Read the model definition and answer for the solid it produces. Units are mm, in the model's axes. Face numbers are marked on the shaded views. Give positions to 0.01 mm unless a question says otherwise; leave off trailing zeros. Order: outer loops, then holes, each group sorted by start corner. A loop starts at its lowest first (then second) coordinate and runs counter-clockwise, first axis right, second up. Notation, with made-up numbers: (46, -5.5) - (99, -5.5) arc R20 ccw to (99, 3.5) - close; hole circle Ø10 at (53.25, 16.25). An arc over 180 degrees is marked (long way). Answer as CSV lines item,"result". Start each with the question number.
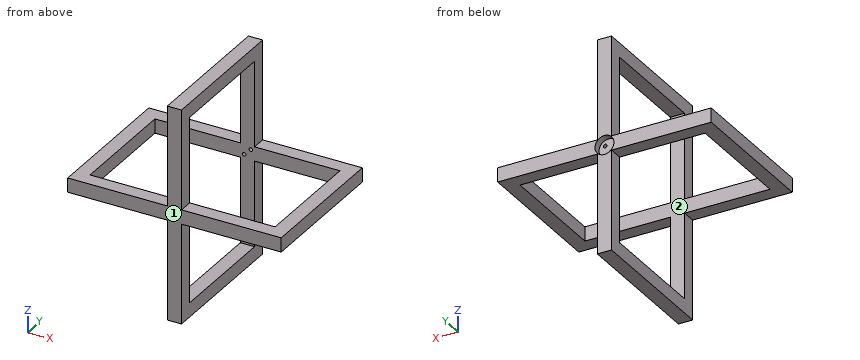
from build123d import *

# Parameters (mm, degrees)
SKETCH1_W                        = 900
SKETCH1_H                        = 600
SKETCH1_W_2                      = 780
SKETCH1_H_2                      = 480
BOSS_EXTRUDE1_DEPTH              = 30
SKETCH2_W                        = 900
SKETCH2_H                        = 600
SKETCH2_W_2                      = 780
SKETCH2_H_2                      = 480
BOSS_EXTRUDE2_DEPTH              = 30
SKETCH3_R                        = 40
CUT_EXTRUDE1_DEPTH               = 30
BLIND_DOWEL_HOLE_0_SIZE_MM_D     = 15
BLIND_DOWEL_HOLE_0_SIZE_MM_DEPTH = 100
BLIND_DOWEL_HOLE_0_SIZE_MM_TIP   = 4.506454643


with BuildPart() as part:
    # Sketch1 → Boss-Extrude1 (new, symmetric)
    with BuildSketch(Plane.XY):
        Rectangle(SKETCH1_W, SKETCH1_H)
        Rectangle(SKETCH1_W_2, SKETCH1_H_2, mode=Mode.SUBTRACT)
    extrude(amount=BOSS_EXTRUDE1_DEPTH, both=True)

    # Sketch2 → Boss-Extrude2 (add, symmetric)
    with BuildSketch(Plane(origin=(0, 0, 0), x_dir=(0, 0, -1), z_dir=(1, 0, 0))):
        Rectangle(SKETCH2_W, SKETCH2_H)
        Rectangle(SKETCH2_W_2, SKETCH2_H_2, mode=Mode.SUBTRACT)
    extrude(amount=BOSS_EXTRUDE2_DEPTH, both=True)

    # Sketch3 → Cut-Extrude1 (cut)
    with BuildSketch(Plane(origin=(0, 300, 0), x_dir=(1, 0, 0), z_dir=(0, 1, 0))):
        with Locations(Location((0, 0, 0), (0, 0, 270))):
            Circle(SKETCH3_R)
    extrude(amount=-CUT_EXTRUDE1_DEPTH, mode=Mode.SUBTRACT)

    # Blind dowel hole 0 (size mm)
    with Locations(Plane(origin=(0, 270, 0), x_dir=(1, 0, 0), z_dir=(0, 1, 0))):
        with Locations((-14.142135624, 14.142135624), (14.142135624, -14.142135624)):
            Hole(BLIND_DOWEL_HOLE_0_SIZE_MM_D / 2, depth=BLIND_DOWEL_HOLE_0_SIZE_MM_DEPTH)
            with Locations((0, 0, -(BLIND_DOWEL_HOLE_0_SIZE_MM_DEPTH + BLIND_DOWEL_HOLE_0_SIZE_MM_TIP / 2))):  # 118° drill point
                Cone(0, BLIND_DOWEL_HOLE_0_SIZE_MM_D / 2, BLIND_DOWEL_HOLE_0_SIZE_MM_TIP, mode=Mode.SUBTRACT)


solid = part.part
(1) Section C-C, the plane y = 167 is taken. Write down the section's boundary in (x, z).
(2) Straight lines are drawn through the part: line 1 (Z direction, x = 19, y = 218.5); line 2 (X direction, y = 276, z = 0); line 3 (Z direction, x = 395, y = -248.5). For each, find the intervals that lie inside material, in ascending order. Write a range as [from, to].
(3) Section A-A, the plane z = -217 is taken. Write down the section's boundary in (x, y), and give its area (3 significant figures).
(4) Determine the mould class of the marked faces 1 and 2 for opening direction X: released by +X, released by -X, zero draft, split by the parting line, or undercut.
(5) Section B-B, the plane x = 252 is taken. Write down the section's boundary in (y, z).
Checks:
1,outline,"(-450, -30) - (-390, -30) - (-390, 30) - (-450, 30) - close; (-30, -450) - (30, -450) - (30, -390) - (-30, -390) - close; (-30, 390) - (30, 390) - (30, 450) - (-30, 450) - close; (390, -30) - (450, -30) - (450, 30) - (390, 30) - close"
2,line 1,"z = [-450, -390], [390, 450]"
2,line 2,"x = [-450, -40], [40, 450]"
2,line 3,"z = [-30, 30]"
3,outline,"(-30, -300) - (30, -300) - (30, -240) - (-30, -240) - close; (-30, 240) - (30, 240) - (30, 300) - (-30, 300) - close"
3,area,"7,200 mm²"
4,face 1,"zero draft"
4,face 2,"undercut"
5,outline,"(-300, -30) - (-240, -30) - (-240, 30) - (-300, 30) - close; (240, -30) - (300, -30) - (300, 30) - (240, 30) - close"
